Source: CAD feature listing. Evaluate the final solid. Frame: model axes, mm. A direction names the side the tool comes from. Give positions to 0.01 mm unless a question says otherwise; leave off trailing zeros. Order: outer loops, then holes, each group sorted by start corner. A loop starts at its lowest first (then second) coordinate and runs counter-clockwise, first axis right, second up. Notation, with made-up numbers: M -12,48.5 L -7,48.5 A23 ccw -7,84.5 Z; hole C -32.5,13.5 d6. An arc over 180 degrees is marked long. Return JSON: item names as keys, results as strings.
from build123d import *

# Parameters (mm, degrees)
SKETCH1_W           = 25
SKETCH1_H           = 18
SKETCH1_R           = 1.5
BOSS_EXTRUDE1_DEPTH = 3
SKETCH2_W           = 25
SKETCH2_H           = 28
SKETCH2_R           = 2.1
BOSS_EXTRUDE2_DEPTH = 3
SKETCH3_R           = 1.75
BOSS_EXTRUDE3_DEPTH = 3


with BuildPart() as part:
    # Sketch1 → Boss-Extrude1 (new body)
    with BuildSketch(Plane.XY):
        Rectangle(SKETCH1_W, SKETCH1_H)
        with Locations((-9.5, 4.5)):
            Circle(SKETCH1_R, mode=Mode.SUBTRACT)
        with Locations((9.5, 4.5)):
            Circle(SKETCH1_R, mode=Mode.SUBTRACT)
        with Locations((9.5, -4.5)):
            Circle(SKETCH1_R, mode=Mode.SUBTRACT)
        with Locations((-9.5, -4.5)):
            Circle(SKETCH1_R, mode=Mode.SUBTRACT)
    extrude(amount=BOSS_EXTRUDE1_DEPTH)

    # Sketch2 → Boss-Extrude2 (add)
    with BuildSketch(Plane(origin=(0, 9, 0), x_dir=(1, 0, 0), z_dir=(0, 1, 0))):
        with Locations((0, 11)):
            Rectangle(SKETCH2_W, SKETCH2_H)
        with Locations(Location((0, 15, 0), (0, 0, 270))):
            Circle(SKETCH2_R, mode=Mode.SUBTRACT)
    extrude(amount=BOSS_EXTRUDE2_DEPTH)

    # Sketch3 → Boss-Extrude3 (add)
    with BuildSketch(Plane.ZY.offset(-12.5)):
        with BuildLine():
            Line((0, -9), (0, 7))
            ThreePointArc((0, 7), (-0.585786438, 8.414213562), (-2, 9))
            Line((-2, 9), (-8, 9))
            ThreePointArc((-8, 9), (-9.414213562, 8.414213562), (-10, 7))
            Line((-10, 7), (-10, -9))
            Line((-10, -9), (-25, -9))
            Line((-25, -9), (-25, 12))
            Line((-25, 12), (3, 12))
            Line((3, 12), (3, -9))
            Line((3, -9), (0, -9))
        make_face()
        with Locations((-21, 1.5)):
            Circle(SKETCH3_R, mode=Mode.SUBTRACT)
        with Locations((-13, 1.5)):
            Circle(SKETCH3_R, mode=Mode.SUBTRACT)
    extrude(amount=-BOSS_EXTRUDE3_DEPTH)


solid = part.part
1. Section query D-D (y = 1.5). Return loops of the section in (x, z), then the cut area to 3 significant figures.
Evaluation:
{"outline": "M -12.5,0 L 15.5,0 L 15.5,3 L -12.5,3 Z; M 12.5,-25 L 15.5,-25 L 15.5,-22.75 L 12.5,-22.75 Z; M 12.5,-19.25 L 15.5,-19.25 L 15.5,-14.75 L 12.5,-14.75 Z; M 12.5,-11.25 L 15.5,-11.25 L 15.5,-10 L 12.5,-10 Z", "area": "108 mm^2"}
2. Section query A-A (x = -9.5). Return loops of the section in (y, z), then the cut area to 3 significant figures.
Evaluation:
{"outline": "M -9,0 L -6,0 L -6,3 L -9,3 Z; M -3,0 L 3,0 L 3,3 L -3,3 Z; M 6,0 L 9,0 L 9,-25 L 12,-25 L 12,3 L 6,3 Z", "area": "120 mm^2"}
3. Section query C-C (z = -21). Return loops of the section in (x, y).
Evaluation:
{"outline": "M -12.5,9 L 12.5,9 L 12.5,3.25 L 15.5,3.25 L 15.5,12 L -12.5,12 Z; M 12.5,-9 L 15.5,-9 L 15.5,-0.25 L 12.5,-0.25 Z"}
4. Section query B-B (y = -7.5). Return loops of the section in (x, z).
Evaluation:
{"outline": "M -12.5,0 L 15.5,0 L 15.5,3 L -12.5,3 Z; M 12.5,-25 L 15.5,-25 L 15.5,-10 L 12.5,-10 Z"}
5. Set-up query: faces 4 (the face through (-1.278, 10.479, -16.666)), 5 (the face through (14, -1, -10)), 6 (the face through (12.5, 8.5, -0.4)). Return all of +Z, -Z, +X, -X, +Y, -Y with unobstructed straight access to the full face (end or side cutting, diameter ignored); none if empty.
Evaluation:
{"face 4": "+Y, -Y", "face 5": "+X, -X, -Y", "face 6": "-Z, -X, -Y"}
6. Draft query along X for faces 1 (the face through (-12.5, 9.2, -5.7)), 2 (the face through (13.98, 1.58, -22.75)), 3 (the face through (-11, -4.43, 1.48)). Return one class per face: pulls with the +X half, pulls with the -X half, needs draft (parallel to the pull), parting line crosses it, or undercut.
Evaluation:
{"face 1": "pulls with the -X half", "face 2": "needs draft", "face 3": "undercut"}
7. First-contact query: pin 1 (5 mm diameter, centred on x = -9.5, y = -4.5, fed in from -Z); pin 2 (5 mm diameter, centred on y = 2, z = -16.5, fed in from -X); pin 3 (6 mm diameter, centred on x = 0.5, z = -12, fed in from -Y). Flat tips, straight axial feed; report the tip coordinate or a pass-through.
Evaluation:
{"pin 1": "stops at z = 0", "pin 2": "stops at x = 12.5", "pin 3": "stops at y = 9"}
8. Ray query, probe 1 along Y at (x, z) = (9.5, 1.05); probe 2 along Y at (x, z) = (13.6, -21); probe 3 along Z at (x, y) = (13, 0). Return the intervals inside material, ascending.
Evaluation:
{"probe 1": "y = -9 to -6, -3 to 3, 6 to 12", "probe 2": "y = -9 to -0.25, 3.25 to 12", "probe 3": "z = -25 to -21.9, -20.1 to -13.9, -12.1 to -10, 0 to 3"}
